CAD build for the part. Positions are in the model's coordinates, mm. A direction names the side the tool comes from. Round coordinates to 2 decimals unless told otherwise and drop trailing zeros. Write each loop counter-clockwise with the first axis right and the second up, starting at its lowest first coordinate (ties: lowest second). Pieces come first, ordered by that corner, then holes. Notation, with made-up numbers: (49.5, 3) - (88.5, 3) arc R11 cw to (88.5, 11) - close; hole circle Ø10 at (2, -24). An arc over 180 degrees is marked (long way). Answer in a Markdown table with one row per item.
```python
from build123d import *

# Parameters (mm, degrees)
SKETCH_1_R      = 25
EXTRUDE_1_DEPTH = 55
SKETCH_2_R      = 22.5
EXTRUDE_2_DEPTH = 25
EXTRUDE_START   = 25
SKETCH_3_R      = 22.5
EXTRUDE_3_DEPTH = 25
CHAMFER_1_SIZE  = 1


with BuildPart() as part:
    # 草图1 → 凸台-拉伸1 (new, symmetric)
    with BuildSketch(Plane.XY):
        Circle(SKETCH_1_R)
    extrude(amount=EXTRUDE_1_DEPTH, both=True)

    # 草图2 → 凸台-拉伸2 (add)
    with BuildSketch(Plane.XY.offset(55)):
        Circle(SKETCH_2_R)
    extrude(amount=EXTRUDE_2_DEPTH)

    # 草图3 → 凸台-拉伸3 (add)
    with BuildSketch(Plane(origin=(0, 0, -55), x_dir=(-1, 0, 0), z_dir=(0, 0, -1)).offset(EXTRUDE_START)):
        with Locations(Location((0, 0, 0), (0, 0, 180))):
            Circle(SKETCH_3_R)
    extrude(amount=-EXTRUDE_3_DEPTH)

    # 倒角1
    chamfer_1_edges = [part.edges().sort_by_distance(p)[0] for p in [
        (-22.5, 0, -80),
        (-22.5, 0, 80),
    ]]
    chamfer(chamfer_1_edges, length=CHAMFER_1_SIZE)


solid = part.part
```
Q1. 3-axis set-ups, long thin cutter, end or side, ignore diameter. For faces 1 (the flat face through (-22.34, 3.82, 55)), 2 (the flat face through (0, 0, 80)), 3 (the cylindrical face through (10.382, 19.961, -67.168)): which of +Z, -Z, +X, -X, +Y, -Y reach the whole face in a straight line?
Computed:
| item | result |
|---|---|
| face 1 | +Z |
| face 2 | +Z, +X, -X, +Y, -Y |
| face 3 | -Z |
Q2. Saw through at A-A on x = 0. List the corners of the cut face in (y, z).
Computed:
| item | result |
|---|---|
| outline | (-25, -55) - (-22.5, -55) - (-22.5, -79) - (-21.5, -80) - (21.5, -80) - (22.5, -79) - (22.5, -55) - (25, -55) - (25, 55) - (22.5, 55) - (22.5, 79) - (21.5, 80) - (-21.5, 80) - (-22.5, 79) - (-22.5, 55) - (-25, 55) - close |
Q3. Saw through at C-C on z = 43. List the corners of the cut face in (x, y).
Computed:
| item | result |
|---|---|
| outline | circle Ø50 at (0, 0) |
Q4. Drill centre lines: line 1 (Y direction, x = 0, z = 46); line 2 (Z direction, x = 21.5, y = 7.5); line 3 (X direction, y = 15.5, z = -11). Where is each one in solid material? Low to high.
Computed:
| item | result |
|---|---|
| line 1 | y = -25 to 25 |
| line 2 | z = -55 to 55 |
| line 3 | x = -19.62 to 19.62 |
Q5. Flat gauge pins, fed straight in: pin 1 (2 mm diameter, centred on y = -7, z = -7.5, fed in from -X); pin 2 (12 mm diameter, centred on y = 6.5, z = 16.5, fed in from -X) (3 decimals); pin 3 (8 mm diameter, centred on x = 7, z = 33, fed in from -Y). Where does each tip first touch, or does it go through?
Computed:
| item | result |
|---|---|
| pin 1 | stops at x = -24.27 |
| pin 2 | stops at x = -24.995 |
| pin 3 | stops at y = -24.82 |
